from build123d import *

# Parameters (mm, degrees)
SKETCH_1_R      = 75
SKETCH_1_R_2    = 9
SKETCH_1_R_3    = 23
EXTRUDE_1_DEPTH = 15
SKETCH_2_R      = 42.5
SKETCH_2_R_2    = 23
EXTRUDE_2_DEPTH = 3


with BuildPart() as part:
    # 草图1 → 凸台-拉伸1 (new body)
    with BuildSketch(Plane(origin=(0, 0, 0), x_dir=(1, 0, 0), z_dir=(0, 1, 0))):
        with Locations(Location((0, 0, 0), (0, 0, 270))):
            Circle(SKETCH_1_R)
        with Locations(Location((0, 55, 0), (0, 0, 270))):
            Circle(SKETCH_1_R_2, mode=Mode.SUBTRACT)
        with Locations(Location((55, 0, 0), (0, 0, 270))):
            Circle(SKETCH_1_R_2, mode=Mode.SUBTRACT)
        with Locations(Location((0, -55, 0), (0, 0, 270))):
            Circle(SKETCH_1_R_2, mode=Mode.SUBTRACT)
        with Locations(Location((-55, 0, 0), (0, 0, 270))):
            Circle(SKETCH_1_R_2, mode=Mode.SUBTRACT)
        with Locations(Location((0, 0, 0), (0, 0, 270))):
            Circle(SKETCH_1_R_3, mode=Mode.SUBTRACT)
    extrude(amount=EXTRUDE_1_DEPTH)

    # 草图2 → 凸台-拉伸2 (add)
    with BuildSketch(Plane(origin=(0, 15, 0), x_dir=(1, 0, 0), z_dir=(0, 1, 0))):
        with Locations(Location((0, 0, 0), (0, 0, 270))):
            Circle(SKETCH_2_R)
        with Locations(Location((0, 0, 0), (0, 0, 270))):
            Circle(SKETCH_2_R_2, mode=Mode.SUBTRACT)
    extrude(amount=EXTRUDE_2_DEPTH)


solid = part.part
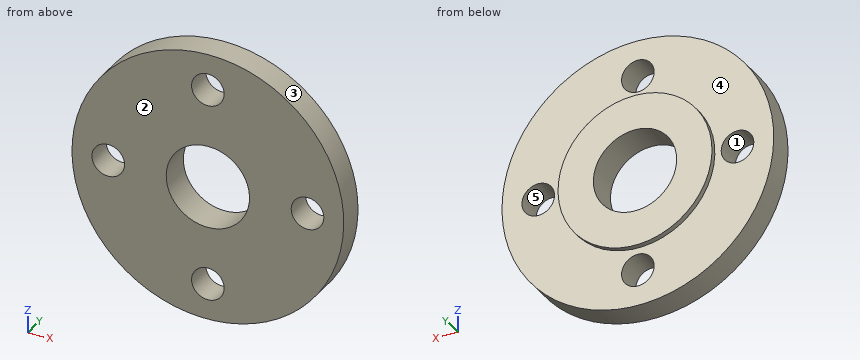
For this review, take the finished solid that the model builds, in its own axes (mm). Face numbers are marked on the shaded views. A direction names the side the tool comes from. Coordinates: 2 decimals unless noted, no trailing zeros. Order: outer loops, then holes, each group sorted by start corner. A loop starts at its lowest first (then second) coordinate and runs counter-clockwise, first axis right, second up. Notation, with made-up numbers: (68.25, 20.25) - (101.25, 20.25) arc R16 cw to (101.25, 25.25) - close; hole circle Ø1 at (-33, -35). An arc over 180 degrees is marked (long way). Answer as CSV lines item,"result". Start each with the question number.
1) Add section A-A (x = 0). State the section outline as (y, z) points.
2) To check wall thickness, follow line 1 along X through (y, z) = (9.5, 0); line 2 along Y through (x, z) = (-60.5, 43); line 3 along X through (y, z) = (3.25, 2). State the ranges of each line that lie inside material, in increasing order. Write a range as [from, to].
3) Add section B-B (z = 0). State the section outline as (x, y) points.
4) Machinability: for the marked faces 4 and 5, which of the approach directions +Z, -Z, +X, -X, +Y, -Y give a long, thin tool a straight path to every point of the face, cutting with its end or side? Answer none if there is none.
5) Draft analysis for pull direction Z (two halves, no side actions). For the marked faces 1, 2 and 3, state which applies: +Z half, -Z half, draft (parallel to the pull), parting line (faces both ways), or undercut.
6) Add section D-D (x = 57). State the section outline as (y, z) points.
7) Insertion check: P1, Ø5, axis at x = -35.5, y = 10, coming from the +Z side; P2, Ø6, axis at x = 24.5, y = 3.5, coming from the +Z side; P3, Ø5, axis at x = 10.5, y = 11, coming from the -Z side. Each pin has a flat end and moves straight along its axis. Give the tip position at first contact, or say it passes through.
8) Add section C-C (z = 52). State the section outline as (x, y) points, then the cut area to 3 significant figures.
Result:
1,outline,"(0, -75) - (15, -75) - (15, -64) - (0, -64) - close; (0, -46) - (15, -46) - (15, -42.5) - (18, -42.5) - (18, -23) - (0, -23) - close; (0, 23) - (18, 23) - (18, 42.5) - (15, 42.5) - (15, 46) - (0, 46) - close; (0, 64) - (15, 64) - (15, 75) - (0, 75) - close"
2,line 1,"[-75, -64], [-46, -23], [23, 46], [64, 75]"
2,line 2,"[0, 15]"
2,line 3,"[-74.97, -63.77], [-46.23, -22.91], [22.91, 46.23], [63.77, 74.97]"
3,outline,"(-75, 0) - (-64, 0) - (-64, 15) - (-75, 15) - close; (-46, 0) - (-23, 0) - (-23, 18) - (-42.5, 18) - (-42.5, 15) - (-46, 15) - close; (23, 0) - (46, 0) - (46, 15) - (42.5, 15) - (42.5, 18) - (23, 18) - close; (64, 0) - (75, 0) - (75, 15) - (64, 15) - close"
4,face 4,"+Y"
4,face 5,"+Y, -Y"
5,face 1,"undercut"
5,face 2,"draft"
5,face 3,"parting line"
6,outline,"(0, -48.74) - (15, -48.74) - (15, -8.77) - (0, -8.77) - close; (0, 8.77) - (15, 8.77) - (15, 48.74) - (0, 48.74) - close"
7,P1,"z = 67.35"
7,P2,"z = 71.85"
7,P3,"z = -74.57"
8,outline,"(-54.05, 0) - (-8.49, 0) - (-8.49, 15) - (-54.05, 15) - close; (8.49, 0) - (54.05, 0) - (54.05, 15) - (8.49, 15) - close"
8,area,"1,370 mm^2"
